Part model, mm, in its own coordinate system. Give positions to 0.01 mm unless a question says otherwise; leave off trailing zeros. Write each loop counter-clockwise with the first axis right and the second up, starting at its lowest first coordinate (ties: lowest second). Pieces come first, ordered by that corner, then holes. Notation, with made-up numbers: M -19,-28.5 L 13,-28.5 A23 ccw 13,-11.5 Z; hole C 7,46 d10. An arc over 180 degrees is marked long. Use CSV: the item, a comma, the result in double quotes. Start each with the question number.
Item 1: Pin check, flat tips, straight feed: pin 1 (3 mm diameter, centred on x = -64.5, y = -1.5, fed in from -Z); pin 2 (3 mm diameter, centred on x = 58, y = 2.5, fed in from +Z); pin 3 (4 mm diameter, centred on x = -58.5, y = 4, fed in from -Z). Stop position of each tip, or through.
Item 2: Drill centre lines: line 1 (X direction, y = -3.5, z = 0); line 2 (X direction, y = -3.5, z = -35.5); line 3 (Z direction, x = -83.5, y = 3.25) (3 decimals). Where is each one in solid material? Low to high. Write a range as [from, to].
Item 3: Cut at B-B (y = 0.5). List the corners of the cut face in (x, z).
Item 4: Cut at C-C (x = -79). List the corners of the cut face in (y, z), then the cut area to 3 significant figures.
Item 5: Cut at A-A (z = 0). List the corners of the cut face in (x, y).
Item 6: Cut at D-D (z = -67). List the corners of the cut face in (x, y).
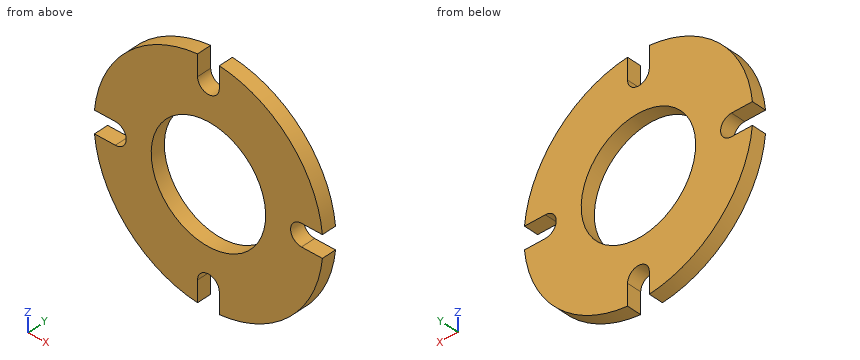
from build123d import *

# Parameters (mm, degrees)
DISK_PROFILE_SKETCH_R       = 50
SLOTTED_DISK_200X12_5_DEPTH = 6.25


with BuildPart() as part:
    # Disk Profile Sketch → Slotted Disk Ø200x12.5 (new, symmetric)
    with BuildSketch(Plane(origin=(0, 0, 0), x_dir=(1, 0, 0), z_dir=(0, 1, 0))):
        with BuildLine():
            Line((-9.5, 81.3), (-9.5, 99.547727247))
            ThreePointArc((-9.5, 99.547727247), (-70.710678119, 70.710678119), (-99.547727247, 9.5))
            Line((-99.547727247, 9.5), (-81.3, 9.5))
            ThreePointArc((-81.3, 9.5), (-71.8, 0), (-81.3, -9.5))
            Line((-81.3, -9.5), (-99.547727247, -9.5))
            ThreePointArc((-99.547727247, -9.5), (-70.710678119, -70.710678119), (-9.5, -99.547727247))
            Line((-9.5, -99.547727247), (-9.5, -81.3))
            ThreePointArc((-9.5, -81.3), (0, -71.8), (9.5, -81.3))
            Line((9.5, -81.3), (9.5, -99.547727247))
            ThreePointArc((9.5, -99.547727247), (70.710678119, -70.710678119), (99.547727247, -9.5))
            Line((99.547727247, -9.5), (81.3, -9.5))
            ThreePointArc((81.3, -9.5), (71.8, 0), (81.3, 9.5))
            Line((81.3, 9.5), (99.547727247, 9.5))
            ThreePointArc((99.547727247, 9.5), (70.710678119, 70.710678119), (9.5, 99.547727247))
            Line((9.5, 99.547727247), (9.5, 81.3))
            ThreePointArc((9.5, 81.3), (0, 71.8), (-9.5, 81.3))
        make_face()
        with Locations(Location((0, 0, 0), (0, 0, 270))):
            Circle(DISK_PROFILE_SKETCH_R, mode=Mode.SUBTRACT)
    extrude(amount=SLOTTED_DISK_200X12_5_DEPTH, both=True)


solid = part.part
Worked answers:
1,pin 1,"stops at z = -77.66"
1,pin 2,"stops at z = 82.51"
1,pin 3,"stops at z = -82.51"
2,line 1,"x = [-71.8, -50], [50, 71.8]"
2,line 2,"x = [-93.49, -35.21], [35.21, 93.49]"
2,line 3,"z = [-55.025, -9.5], [9.5, 55.025]"
3,outline,"M -99.55,-9.5 A100 ccw -9.5,-99.55 L -9.5,-81.3 A9.5 cw 9.5,-81.3 L 9.5,-99.55 A100 ccw 99.55,-9.5 L 81.3,-9.5 A9.5 cw 81.3,9.5 L 99.55,9.5 A100 ccw 9.5,99.55 L 9.5,81.3 A9.5 cw -9.5,81.3 L -9.5,99.55 A100 ccw -99.55,9.5 L -81.3,9.5 A9.5 cw -81.3,-9.5 Z; hole C 0,0 d100"
4,outline,"M -6.25,-61.31 L 6.25,-61.31 L 6.25,-9.22 L -6.25,-9.22 Z; M -6.25,9.22 L 6.25,9.22 L 6.25,61.31 L -6.25,61.31 Z"
4,area,"1,300 mm^2"
5,outline,"M -71.8,-6.25 L -50,-6.25 L -50,6.25 L -71.8,6.25 Z; M 50,-6.25 L 71.8,-6.25 L 71.8,6.25 L 50,6.25 Z"
6,outline,"M -74.24,-6.25 L 74.24,-6.25 L 74.24,6.25 L -74.24,6.25 Z"
